```python
from build123d import *

# Parameters (mm, degrees)
BASE_PLATE_PROFILE_SKETCH_R   = 30
BASE_PLATE_PROFILE_SKETCH_R_2 = 13
BASE_PLATE_DEPTH              = 20
BASE_SLOT_CUT_REACH           = 100.874
BASE_SLOT_SKETCH_W            = 35
BASE_SLOT_SKETCH_H            = 10
BORE_CUT_REACH                = 86.119
BORE_SKETCH_W                 = 30
BORE_SKETCH_H                 = 10
UPRIGHT_BLOCK_DEPTH           = 30
UPRIGHT_BLOCK_DEPTH_BACK      = 30
UPRIGHT_POCKET_SKETCH_W       = 40
UPRIGHT_POCKET_SKETCH_H       = 20
UPRIGHT_POCKET_CUT_DEPTH      = 20


with BuildPart() as part:
    # Base Plate Profile Sketch → Base Plate (new body)
    # profile 1 of 2: a face of its own
    with BuildSketch(Plane(origin=(0, 0, 0), x_dir=(0, 0, -1), z_dir=(0, -1, 0))):
        with BuildLine():
            Line((76, 30), (0, 30))
            ThreePointArc((0, 30), (21.213203436, 21.213203436), (30, 0))
            ThreePointArc((30, 0), (21.213203436, -21.213203436), (0, -30))
            Line((0, -30), (76, -30))
            Line((76, -30), (76, 30))
        make_face()
    # profile 2 of 2: a face of its own
    with BuildSketch(Plane(origin=(0, 0, 0), x_dir=(0, 0, -1), z_dir=(0, -1, 0))):
        Circle(BASE_PLATE_PROFILE_SKETCH_R)
        with Locations(Location((0, 0, 0), (0, 0, 180))):
            Circle(BASE_PLATE_PROFILE_SKETCH_R_2, mode=Mode.SUBTRACT)
    extrude(amount=-BASE_PLATE_DEPTH)

    # Base Slot Sketch → Base Slot Cut (cut, up to next)
    with BuildSketch(Plane(origin=(30, 0, 0), x_dir=(0, 0, -1), z_dir=(1, 0, 0)), mode=Mode.PRIVATE) as base_slot_cut_sk1:
        with Locations((43.5, 5)):
            Rectangle(BASE_SLOT_SKETCH_W, BASE_SLOT_SKETCH_H)
    base_slot_cut_tool1 = extrude(base_slot_cut_sk1.sketch, amount=-BASE_SLOT_CUT_REACH, mode=Mode.PRIVATE) & part.part
    add(base_slot_cut_tool1.solids().sort_by_distance((30, 5, -43.5))[0], mode=Mode.SUBTRACT)

    # Bore Sketch → Bore Cut (cut, up to next)
    with BuildSketch(Plane(origin=(0, 20, 0), x_dir=(1, 0, 0), z_dir=(0, 1, 0)), mode=Mode.PRIVATE) as bore_cut_sk1:
        with Locations((0, 71)):
            Rectangle(BORE_SKETCH_W, BORE_SKETCH_H)
    bore_cut_tool1 = extrude(bore_cut_sk1.sketch, amount=-BORE_CUT_REACH, mode=Mode.PRIVATE) & part.part
    add(bore_cut_tool1.solids().sort_by_distance((0, 20, -71))[0], mode=Mode.SUBTRACT)

    # Upright Block Profile Sketch → Upright Block (add, two sides: drawn at the far end of the back side and taken through both)
    with BuildSketch(Plane(origin=(0, 0, 0), x_dir=(0, 0, -1), z_dir=(1, 0, 0)).offset(-UPRIGHT_BLOCK_DEPTH_BACK)):
        Polygon((0, 20), (0, 40), (30, 40), (40, 20), align=None)
    extrude(amount=UPRIGHT_BLOCK_DEPTH + UPRIGHT_BLOCK_DEPTH_BACK)

    # Upright Pocket Sketch → Upright Pocket Cut (cut)
    with BuildSketch(Plane(origin=(0, 40, 0), x_dir=(1, 0, 0), z_dir=(0, 1, 0))):
        with Locations((0, 10)):
            Rectangle(UPRIGHT_POCKET_SKETCH_W, UPRIGHT_POCKET_SKETCH_H)
    extrude(amount=-UPRIGHT_POCKET_CUT_DEPTH, mode=Mode.SUBTRACT)


solid = part.part
```
Geometry: final body of the model. Coordinates: model frame, mm. A direction names the side the tool comes from. Coordinates: 2 decimals unless noted, no trailing zeros. Order: outer loops, then holes, each group sorted by start corner. A loop starts at its lowest first (then second) coordinate and runs counter-clockwise, first axis right, second up. Notation, with made-up numbers: (33, -19.75) -> (79, -19.75) arc R18 cw to (79, -3.75) -> close; hole circle Ø1 at (-5, 85.25). An arc over 180 degrees is marked (long way). Write item = value, one per line.
(1) Cut plane B-B on x = 0. Return loops of the section in (y, z), plus the area to 3 significant figures.
Solved:
outline = (0, -66) -> (20, -66) -> (20, -40) -> (40, -30) -> (40, -20) -> (20, -20) -> (20, -13) -> (0, -13) -> (0, -26) -> (10, -26) -> (10, -61) -> (0, -61) -> close; (0, 13) -> (20, 13) -> (20, 30) -> (0, 30) -> close
area = 1,350 mm²
(2) Cut plane D-D on x = 18. Return loops of the section in (y, z), plus the area to 3 significant figures.
Solved:
outline = (0, -76) -> (20, -76) -> (20, -40) -> (40, -30) -> (40, -20) -> (20, -20) -> (20, 24) -> (0, 24) -> (0, -26) -> (10, -26) -> (10, -61) -> (0, -61) -> close
area = 1,950 mm²
(3) Pin query (flat end, axial travel): pin 1 Ø8 at (x, y) = (-23, 27.5) entering from +Z; pin 2 Ø12 at (x, y) = (-7.5, 22) entering from +Z; pin 3 Ø11 at (x, y) = (14, 3.5) entering from +Z. Return the tip coordinate at first contact, or that it passes through.
Solved:
pin_1 = 0
pin_2 = 29.94
pin_3 = 28.77
(4) Cut plane A-A on y = 4. Return loops of the section in (x, z), plus the area to 3 significant figures.
Solved:
outline = (-30, -76) -> (-15, -76) -> (-15, -66) -> (15, -66) -> (15, -76) -> (30, -76) -> (30, -61) -> (-30, -61) -> close; (-30, -26) -> (30, -26) -> (30, 0) arc R30 ccw to (-30, 0) -> close; hole circle Ø26 at (0, 0)
area = 3,040 mm²
(5) Pull-direction query (Z, two-part tool) for faces 6 (the flat face through (-25, 30, 0)), 7 (the flat face through (0, 10, -43)), 8 (the flat face through (-15, 10, -71)); classes: pulls with the +Z half, pulls with the -Z half, needs draft (parallel to the pull), parting line crosses it, or undercut.
Solved:
face_6 = pulls with the +Z half
face_7 = undercut
face_8 = needs draft
(6) Access query for faces 1 (the cylindrical face through (7.91, 9.86, -10.316)), 2 (the flat face through (20, 30, -10)), 3 (the flat face through (0, 10, -66)), 4 (the flat face through (-30, 20, -30)), 5 (the flat face through (0, 5, -61)). Directions: +Z, -Z, +X, -X, +Y, -Y. A direction counts if a zero-diameter tool reaches every point of the face in a straight line with its end or side. Return the directions, or none.
Solved:
face_1 = +Y, -Y
face_2 = +Z, +Y
face_3 = -Z, +Y, -Y
face_4 = +Z, -Z, -X, +Y, -Y
face_5 = +X, -X, -Y
(7) Line query: line 1 (X direction, y = 12, z = 0); line 2 (X direction, y = 9, z = -71); line 3 (Y direction, x = 1.5, z = 13.5). Output: solid intervals per line, ascending.
Solved:
line_1 = -30 to -13, 13 to 30
line_2 = -30 to -15, 15 to 30
line_3 = 0 to 20
(8) Cut plane C-C on y = 16. Return loops of the section in (x, z), plus the area to 3 significant figures.
Solved:
outline = (-30, -76) -> (-15, -76) -> (-15, -66) -> (15, -66) -> (15, -76) -> (30, -76) -> (30, 0) arc R30 ccw to (-30, 0) -> close; hole circle Ø26 at (0, 0)
area = 5,140 mm²
